Build history of the part. All positions in model axes, mm. A direction names the side the tool comes from. Round coordinates to 2 decimals unless told otherwise and drop trailing zeros. Loops run counter-clockwise (first coordinate to the right, second up) from the corner with the lowest first, then second, coordinate; pieces in that order, holes last. Notation, with made-up numbers: (24.5, 34) - (47.5, 34) arc R33 cw to (47.5, 70) - close; hole circle Ø11 at (2, 4). An arc over 180 degrees is marked (long way). Use a Markdown table: item, result.
from build123d import *

# Parameters (mm, degrees)
SKETCH1_R           = 6
BOSS_EXTRUDE1_DEPTH = 4
SKETCH2_R           = 4
BOSS_EXTRUDE2_DEPTH = 31
SKETCH3_R           = 2
BOSS_EXTRUDE3_DEPTH = 1.5
CUT_EXTRUDE1_DEPTH  = 4
CHAMFER1_SIZE       = 0.5
CHAMFER2_SIZE       = 0.2
FILLET1_R           = 1


with BuildPart() as part:
    # Sketch1 → Boss-Extrude1 (new, symmetric)
    with BuildSketch(Plane(origin=(0, 0, 0), x_dir=(1, 0, 0), z_dir=(0, 1, 0))):
        with Locations(Location((0, 0, 0), (0, 0, 270))):
            Circle(SKETCH1_R)
    extrude(amount=BOSS_EXTRUDE1_DEPTH, both=True)

    # Sketch2 → Boss-Extrude2 (add)
    with BuildSketch(Plane(origin=(0, 4, 0), x_dir=(1, 0, 0), z_dir=(0, 1, 0))):
        with Locations(Location((0, 0, 0), (0, 0, 270))):
            Circle(SKETCH2_R)
    extrude(amount=BOSS_EXTRUDE2_DEPTH)

    # Sketch3 → Boss-Extrude3 (add)
    with BuildSketch(Plane(origin=(0, 35, 0), x_dir=(1, 0, 0), z_dir=(0, 1, 0))):
        with Locations(Location((0, 0, 0), (0, 0, 270))):
            Circle(SKETCH3_R)
    extrude(amount=BOSS_EXTRUDE3_DEPTH)

    # Sketch4 → Cut-Extrude1 (cut)
    with BuildSketch(Plane.XZ.offset(4)):
        Polygon((2.886751346, 0), (1.443375673, 2.5), (-1.443375673, 2.5), (-2.886751346, 0), (-1.443375673, -2.5), (1.443375673, -2.5), align=None)
    extrude(amount=-CUT_EXTRUDE1_DEPTH, mode=Mode.SUBTRACT)

    # Chamfer1
    chamfer1_edges = [part.edges().sort_by_distance(p)[0] for p in [
        (0, -4, -6),
        (0, 35, -4),
    ]]
    chamfer(chamfer1_edges, length=CHAMFER1_SIZE)

    # Chamfer2
    chamfer2_edges = [part.edges().sort_by_distance(p)[0] for p in [
        (0, 4, -6),
    ]]
    chamfer(chamfer2_edges, length=CHAMFER2_SIZE)

    # Fillet1
    fillet1_edges = [part.edges().sort_by_distance(p)[0] for p in [
        (0, 36.5, -2),
    ]]
    fillet(fillet1_edges, radius=FILLET1_R)

    # Sketch5 → Cut-Revolve1 (revolve, cut)
    with BuildSketch(Plane(origin=(0, 0, 0), x_dir=(0, 0, -1), z_dir=(1, 0, 0))):
        Polygon((2.5, 0), (0, 1.443375673), (0, 0), align=None)
    revolve(axis=Axis((0, 0, 0), (0, -1, 0)), mode=Mode.SUBTRACT)


solid = part.part
Q1. Drop flat-ended pins along their axis: pin 1 (2 mm diameter, centred on x = -2, y = 26, fed in from -Z); pin 2 (1 mm diameter, centred on y = 14.5, z = 1.5, fed in from +X); pin 3 (3 mm diameter, centred on x = -3.5, y = 27.5, fed in from -Z). Give the stop position or say it passes through.
Results found:
| item | result |
|---|---|
| pin 1 | stops at z = -3.87 |
| pin 2 | stops at x = 3.87 |
| pin 3 | stops at z = -3.46 |
Q2. Cut at A-A, the plane y = 18. List the corners of the cut face in (x, z), plus the area to 3 significant figures.
Results found:
| item | result |
|---|---|
| outline | circle Ø8 at (0, 0) |
| area | 50.3 mm2 |
Q3. Which spindle directions (+Z, -Z, +X, -X, +Y, -Y) get a long thin tool onto all of the face, cutting with end or side? Do faces 1 (the face through (-3.905, 19.036, -0.867)), 2 (the face through (1.802, 0.201, 5.723)), 3 (the face through (-2.155, -2.028, 1.267)). Say none if no direction does.
Results found:
| item | result |
|---|---|
| face 1 | +Y |
| face 2 | +Y, -Y |
| face 3 | -Y |
Q4. Pull direction X, two halves, no side cores. Call faces 4 (the face through (-1.952, 35.246, -0.434)), 5 (the face through (-2.175, -2.028, -1.233)), 6 (the face through (0, -4, -3)): pulls with the +X half, pulls with the -X half, needs draft (parallel to the pull), parting line crosses it, or undercut.
Results found:
| item | result |
|---|---|
| face 4 | parting line crosses it |
| face 5 | undercut |
| face 6 | needs draft |
Q5. Probe line 1 (Y direction, x = -4.75, z = -0.25); line 2 (Y direction, x = 2, z = 2.75); line 3 (Z direction, x = 1.25, y = -0.5). List the from-to ranges inside material, lowest first.
Results found:
| item | result |
|---|---|
| line 1 | y = -4 to 4 |
| line 2 | y = -4 to 35 |
| line 3 | z = -5.87 to -2.5, 2.5 to 5.87 |
